Here's how the part is built. I have some questions about the finished solid (model axes, mm). Coordinates: 2 decimals unless noted, no trailing zeros. Loops run counter-clockwise (first coordinate to the right, second up) from the corner with the lowest first, then second, coordinate; pieces in that order, holes last. Notation, with made-up numbers: (-21, 51.25) - (9, 51.25) arc R9 cw to (9, 62.25) - close; hole circle Ø10 at (-24.75, -22.75). An arc over 180 degrees is marked (long way). Use a Markdown table: item, result.
```python
from build123d import *

# Parameters (mm, degrees)
EXTRUDE_1_DEPTH     = 8
SKETCH_2_R          = 10
CUT_EXTRUDE_1_DEPTH = 24


with BuildPart() as part:
    # 草图1 → 凸台-拉伸1 (new body)
    with BuildSketch(Plane.XY):
        Polygon((0, 0), (0, 80), (310, 80), (320, 80), (320, 0), align=None)
    extrude(amount=EXTRUDE_1_DEPTH)

    # 草图2 → 切除-拉伸1 (cut)
    with BuildSketch(Plane.XY.offset(8)):
        with Locations((80, 40)):
            Circle(SKETCH_2_R)
        with Locations((160, 40)):
            Circle(SKETCH_2_R)
        with Locations((240, 40)):
            Circle(SKETCH_2_R)
    extrude(amount=-CUT_EXTRUDE_1_DEPTH, mode=Mode.SUBTRACT)


solid = part.part
```
Q1. Please list where these lines run through material, in increasing order: L1, parallel to Y at x = 240, z = 4.25; L2, parallel to X at y = 35, z = 7.25; L3, parallel to X at y = 44, z = 6.75. Write a range as from..to.
Check values:
| item | result |
|---|---|
| L1 | 0..30, 50..80 |
| L2 | 0..71.34, 88.66..151.34, 168.66..231.34, 248.66..320 |
| L3 | 0..70.83, 89.17..150.83, 169.17..230.83, 249.17..320 |
Q2. I want a section at B-B, the plane x = 160. Write out the boundary of the cut face in (y, z), then the cut area to 3 significant figures.
Check values:
| item | result |
|---|---|
| outline | (0, 0) - (30, 0) - (30, 8) - (0, 8) - close; (50, 0) - (80, 0) - (80, 8) - (50, 8) - close |
| area | 480 mm^2 |
Q3. Will these pins go through, and if not, where does the flat tip stop? P1, Ø4, axis at x = 97.5, z = 3, coming from the -Y side; P2, Ø12, axis at x = 80, y = 40, coming from the -Z side.
Check values:
| item | result |
|---|---|
| P1 | y = 0 |
| P2 | through |
Q4. I want a section at C-C, the plane z = 1.75. Write out the boundary of the cut face in (x, y).
Check values:
| item | result |
|---|---|
| outline | (0, 0) - (320, 0) - (320, 80) - (0, 80) - close; hole circle Ø20 at (80, 40); hole circle Ø20 at (160, 40); hole circle Ø20 at (240, 40) |
Q5. I want a section at A-A, the plane y = 40. Write out the boundary of the cut face in (x, z).
Check values:
| item | result |
|---|---|
| outline | (0, 0) - (70, 0) - (70, 8) - (0, 8) - close; (90, 0) - (150, 0) - (150, 8) - (90, 8) - close; (170, 0) - (230, 0) - (230, 8) - (170, 8) - close; (250, 0) - (320, 0) - (320, 8) - (250, 8) - close |
Q6. If we mould it in two halves opening along X, with no side actions, what happens to faces 1 (the face through (162, 58, 8)), 2 (the face through (169.237, 36.17, 4.056)), 3 (the face through (0, 39, 4))? For each: pulls with the +X half, pulls with the -X half, needs draft (parallel to the pull), parting line crosses it, or undercut.
Check values:
| item | result |
|---|---|
| face 1 | needs draft |
| face 2 | undercut |
| face 3 | pulls with the -X half |
